```python
from build123d import *

# Parameters (mm, degrees)
SKETCH1_W                                            = 60
SKETCH1_H                                            = 25
BOSS_EXTRUDE1_DEPTH                                  = 35
SKETCH2_R                                            = 6.5
CUT_EXTRUDE1_DEPTH                                   = 53.440442409
SKETCH3_R                                            = 9
CUT_EXTRUDE2_DEPTH                                   = 10
SKETCH6_W                                            = 9.5
SKETCH6_H                                            = 70
CUT_EXTRUDE3_DEPTH                                   = 1
M4_TAPPED_HOLE1_D                                    = 3.3
M4_TAPPED_HOLE1_DEPTH                                = 12
M4_TAPPED_HOLE1_TIP                                  = 0.991420021
CUT_EXTRUDE4_DEPTH                                   = 7
M5_TAPPED_HOLE1_D                                    = 4.2
M5_TAPPED_HOLE1_DEPTH                                = 14
M5_TAPPED_HOLE1_TIP                                  = 1.2618073
HOLE_SIZE_PER_SOCKET_HEAD_CAP_SCREW_TYPE_D           = 4.5
HOLE_SIZE_PER_SOCKET_HEAD_CAP_SCREW_TYPE_CBORE_D     = 8
HOLE_SIZE_PER_SOCKET_HEAD_CAP_SCREW_TYPE_CBORE_DEPTH = 4
F_6_0_6_DIAMETER_HOLE2_D                             = 6
HOLE_SIZE_PER_SOCKET_HEAD_CAP_SCREW_2_D              = 6.6
HOLE_SIZE_PER_SOCKET_HEAD_CAP_SCREW_2_CBORE_D        = 11
HOLE_SIZE_PER_SOCKET_HEAD_CAP_SCREW_2_CBORE_DEPTH    = 6.8
M4_TAPPED_HOLE2_D                                    = 3.3
M4_TAPPED_HOLE2_DEPTH                                = 15
M4_TAPPED_HOLE2_TIP                                  = 0.991420021
CHAMFER1_SIZE                                        = 1


with BuildPart() as part:
    # Sketch1 → Boss-Extrude1 (new, symmetric)
    with BuildSketch(Plane.XY):
        with Locations((0, 12.5)):
            Rectangle(SKETCH1_W, SKETCH1_H)
    extrude(amount=BOSS_EXTRUDE1_DEPTH, both=True)

    # Sketch2 → Cut-Extrude1 (cut, through all)
    with BuildSketch(Plane(origin=(0, 25, 0), x_dir=(1, 0, 0), z_dir=(0, 1, 0))):
        with Locations(Location((7, 25, 0), (0, 0, 270))):
            Circle(SKETCH2_R)
        with Locations(Location((17, -25, 0), (0, 0, 270))):
            Circle(SKETCH2_R)
        with BuildLine():
            Line((-24.5, 13.25), (-21.5, 13.25))
            ThreePointArc((-21.5, 13.25), (-18.25, 10), (-21.5, 6.75))
            Line((-21.5, 6.75), (-24.5, 6.75))
            ThreePointArc((-24.5, 6.75), (-27.75, 10), (-24.5, 13.25))
        make_face()
        with BuildLine():
            Line((-24.5, -6.75), (-21.5, -6.75))
            ThreePointArc((-21.5, -6.75), (-18.25, -10), (-21.5, -13.25))
            Line((-21.5, -13.25), (-24.5, -13.25))
            ThreePointArc((-24.5, -13.25), (-27.75, -10), (-24.5, -6.75))
        make_face()
    extrude(amount=-CUT_EXTRUDE1_DEPTH, mode=Mode.SUBTRACT)

    # Sketch3 → Cut-Extrude2 (cut)
    with BuildSketch(Plane.XZ):
        with Locations(Location((17, 25, 0), (0, 0, 270))):
            Circle(SKETCH3_R)
        with Locations(Location((7, -25, 0), (0, 0, 270))):
            Circle(SKETCH3_R)
    extrude(amount=-CUT_EXTRUDE2_DEPTH, mode=Mode.SUBTRACT)

    # Sketch6 → Cut-Extrude3 (cut)
    with BuildSketch(Plane(origin=(0, 25, 0), x_dir=(-1, 0, 0), z_dir=(0, 1, 0))):
        with Locations((11.25, 0)):
            Rectangle(SKETCH6_W, SKETCH6_H)
    extrude(amount=-CUT_EXTRUDE3_DEPTH, mode=Mode.SUBTRACT)

    # M4 Tapped Hole1
    with Locations(Plane(origin=(0, 24, 0), x_dir=(-1, 0, 0), z_dir=(0, 1, 0))):
        with Locations((11.25, 4.5), (11.25, -4.5)):
            Hole(M4_TAPPED_HOLE1_D / 2, depth=M4_TAPPED_HOLE1_DEPTH)
            with Locations((0, 0, -(M4_TAPPED_HOLE1_DEPTH + M4_TAPPED_HOLE1_TIP / 2))):  # 118° drill point
                Cone(0, M4_TAPPED_HOLE1_D / 2, M4_TAPPED_HOLE1_TIP, mode=Mode.SUBTRACT)

    # Sketch10 → Cut-Extrude4 (cut)
    with BuildSketch(Plane.XZ):
        with BuildLine():
            Line((-21.5, -16), (-30, -16))
            ThreePointArc((-30, -16), (-36, -10), (-30, -4))
            Line((-30, -4), (-21.5, -4))
            ThreePointArc((-21.5, -4), (-15.5, -10), (-21.5, -16))
        make_face()
        with BuildLine():
            Line((-21.5, 4), (-30, 4))
            ThreePointArc((-30, 4), (-36, 10), (-30, 16))
            Line((-30, 16), (-21.5, 16))
            ThreePointArc((-21.5, 16), (-15.5, 10), (-21.5, 4))
        make_face()
    extrude(amount=-CUT_EXTRUDE4_DEPTH, mode=Mode.SUBTRACT)

    # M5 Tapped Hole1
    with Locations(Plane(origin=(0, 0, -35), x_dir=(-1, 0, 0), z_dir=(0, 0, -1))):
        with Locations((-22.5, 19), (-22.5, 6), (22.5, 19), (22.5, 6)):
            Hole(M5_TAPPED_HOLE1_D / 2, depth=M5_TAPPED_HOLE1_DEPTH)
            with Locations((0, 0, -(M5_TAPPED_HOLE1_DEPTH + M5_TAPPED_HOLE1_TIP / 2))):  # 118° drill point
                Cone(0, M5_TAPPED_HOLE1_D / 2, M5_TAPPED_HOLE1_TIP, mode=Mode.SUBTRACT)

    # Hole size per socket head cap screw type (through all)
    with Locations(Plane.XZ):
        with Locations((-11.25, -4.5), (-11.25, 4.5)):
            CounterBoreHole(HOLE_SIZE_PER_SOCKET_HEAD_CAP_SCREW_TYPE_D / 2, HOLE_SIZE_PER_SOCKET_HEAD_CAP_SCREW_TYPE_CBORE_D / 2, HOLE_SIZE_PER_SOCKET_HEAD_CAP_SCREW_TYPE_CBORE_DEPTH)

    # Ø6.0 (6) Diameter Hole2 (through all)
    with Locations(Plane(origin=(0, 0, 0), x_dir=(-1, 0, 0), z_dir=(0, -1, 0))):
        with Locations((11.5, -25), (11.5, 25)):
            Hole(F_6_0_6_DIAMETER_HOLE2_D / 2)

    # Hole size per socket head cap screw  2 (through all)
    with Locations(Plane(origin=(0, 25, 0), x_dir=(1, 0, 0), z_dir=(0, 1, 0))):
        with Locations((0, -25), (20, 15)):
            CounterBoreHole(HOLE_SIZE_PER_SOCKET_HEAD_CAP_SCREW_2_D / 2, HOLE_SIZE_PER_SOCKET_HEAD_CAP_SCREW_2_CBORE_D / 2, HOLE_SIZE_PER_SOCKET_HEAD_CAP_SCREW_2_CBORE_DEPTH)

    # M4 Tapped Hole2
    with Locations(Plane(origin=(30, 0, 0), x_dir=(0, 0, -1), z_dir=(1, 0, 0))):
        with Locations((0, 15)):
            Hole(M4_TAPPED_HOLE2_D / 2, depth=M4_TAPPED_HOLE2_DEPTH)
            with Locations((0, 0, -(M4_TAPPED_HOLE2_DEPTH + M4_TAPPED_HOLE2_TIP / 2))):  # 118° drill point
                Cone(0, M4_TAPPED_HOLE2_D / 2, M4_TAPPED_HOLE2_TIP, mode=Mode.SUBTRACT)

    # Chamfer1
    chamfer1_edges = [part.edges().sort_by_distance(p)[0] for p in [
        (30, 12.5, 35),
        (-30, 12.5, 35),
        (30, 12.5, -35),
        (-30, 12.5, -35),
    ]]
    chamfer(chamfer1_edges, length=CHAMFER1_SIZE)


solid = part.part
```
Geometry check sheet. Reference: the model listing, model coordinates, mm. A direction names the side the tool comes from. Give positions to 0.01 mm unless a question says otherwise; leave off trailing zeros. Order: outer loops, then holes, each group sorted by start corner. A loop starts at its lowest first (then second) coordinate and runs counter-clockwise, first axis right, second up. Notation, with made-up numbers: (43.5, 13.5) - (90.5, 13.5) arc R12 ccw to (90.5, 36.5) - close; hole circle Ø10 at (20, 82.5). An arc over 180 degrees is marked (long way). Write item = value, one per line. Start each with the question number.
1) Section check B-B (y = 9). Count the separate pieces of the cut face and the enclosed holes in it, then the cut area to 3 significant figures.
2) Draft check along Z on faces 1 (the cylindrical face through (-13.9, 12.2, 26.8)), 2 (the cylindrical face through (-20.497, 6.631, -27.902)), 3 (the flat face through (-9.5, 4, -6.2)), 4 (the flat face through (0, 13, 35)). Enter one of: released by +Z, released by -Z, zero draft, split by the parting line, or undercut.
3) Scan lines: L1, parallel to Z at x = -11.25, y = 2.85; L2, parallel to Z at x = -11.25, y = 9.5; L3, parallel to Y at x = -22.5, z = -26.25. Record each from-to range of solid material in increasing order.
4) Section check D-D (z = -15). Enter the section's corners in (x, y).
5) Gauge pin test, flat ends, axial feed: pin 1 Ø2.5 at (x, y) = (-22.5, 19) entering from -Z; pin 2 Ø6.5 at (x, z) = (-11.25, 4.5) entering from +Y. Record the tip position at first contact, or that the pin passes through.
6) Section check A-A (z = 25). Enter the section's corners in (x, y), then the cut area to 3 significant figures.
7) Section check C-C (x = 18.5). Enter the section's corners in (y, z), then the cut area to 3 significant figures.
8) Access from +Z, -Z, +X, -X, +Y, -Y to the whole of each face (thin tool, end or side, straight path). Record for faces 5 (the flat face through (-26, 3, 4)), 6 (the cylindrical face through (22.4, 16.39, 0.89)), 7 (the cylindrical face through (23.63, 20.77, -27.9)), 8 (the flat face through (-23, 16, -13.25)), 9 (the cylindrical face through (-14.424, 1.972, 2.066)).
Geometry check:
q1.separate_pieces = 1
q1.enclosed_holes = 10
q1.area = 3,430 mm2
q2.face_1 = undercut
q2.face_2 = zero draft
q2.face_3 = undercut
q2.face_4 = released by +Z
q3.L1 = -35 to -27.99, -22.01 to -8.5, -0.5 to 0.5, 8.5 to 22.01, 27.99 to 35
q3.L2 = -35 to -27.99, -22.01 to -6.75, -2.25 to 2.25, 6.75 to 22.01, 27.99 to 35
q3.L3 = 0 to 3.9, 8.1 to 16.9, 21.1 to 25
q4.outline = (-30, 7) - (-18.18, 7) - (-18.18, 0) - (16.7, 0) - (16.7, 18.2) - (14.5, 18.2) - (14.5, 25) - (-6.5, 25) - (-6.5, 24) - (-16, 24) - (-16, 25) - (-30, 25) - close; (23.3, 0) - (30, 0) - (30, 25) - (25.5, 25) - (25.5, 18.2) - (23.3, 18.2) - close
q5.pin_1 = -20.49
q5.pin_2 = 24
q6.outline = (-30, 0) - (-14.5, 0) - (-14.5, 24) - (-16, 24) - (-16, 25) - (-30, 25) - close; (-8.5, 0) - (-3.3, 0) - (-3.3, 18.2) - (-5.5, 18.2) - (-5.5, 25) - (-6.5, 25) - (-6.5, 24) - (-8.5, 24) - close; (3.3, 0) - (8, 0) - (8, 10) - (10.5, 10) - (10.5, 25) - (5.5, 25) - (5.5, 18.2) - (3.3, 18.2) - close; (23.5, 10) - (26, 10) - (26, 0) - (30, 0) - (30, 25) - (23.5, 25) - close
q6.area = 777 mm2
q7.outline = (0, -35) - (25, -35) - (25, -20.29) - (18.2, -20.29) - (18.2, -17.94) - (0, -17.94) - close; (0, -12.06) - (18.2, -12.06) - (18.2, -9.71) - (25, -9.71) - (25, 18.68) - (10, 18.68) - (10, 16.13) - (0, 16.13) - close; (0, 33.87) - (10, 33.87) - (10, 31.32) - (25, 31.32) - (25, 35) - (0, 35) - close; hole circle Ø3.3 at (15, 0)
q7.area = 1,200 mm2
q8.face_5 = -X, -Y
q8.face_6 = +X
q8.face_7 = -Z
q8.face_8 = +Y, -Y
q8.face_9 = -Y
